```python
from build123d import *

# Parameters (mm, degrees)
EXTRUDE_1_DEPTH = 25


with BuildPart() as part:
    # 草图1 → 凸台-拉伸1 (new body)
    with BuildSketch(Plane(origin=(0, 0, 0), x_dir=(1, 0, 0), z_dir=(0, 1, 0))):
        Polygon((-115, 90), (-90, 115), (0, 115), (0, 0), (-115, 0), align=None)
    extrude(amount=EXTRUDE_1_DEPTH)


solid = part.part
```
Input: part model. Units: mm. Frame: model coordinates. Coordinates: 2 decimals unless noted, no trailing zeros. Loops run counter-clockwise (first coordinate to the right, second up) from the corner with the lowest first, then second, coordinate; pieces in that order, holes last. Notation, with made-up numbers: (27.5, -1) -> (55.5, -1) arc R23 ccw to (55.5, 14) -> close; hole circle Ø6 at (-2, 3.25). An arc over 180 degrees is marked (long way). Use a Markdown table: item, result.
1) Cut plane A-A (y = 9.5). Return the cut outline in (x, z), then the cut area to 3 significant figures.
Results found:
| item | result |
|---|---|
| outline | (-115, -90) -> (-90, -115) -> (0, -115) -> (0, 0) -> (-115, 0) -> close |
| area | 12,900 mm2 |
2) Material intervals for line 1 along X through (y, z) = (9, -97.5); line 2 along Z through (x, y) = (-107.5, 23.75); line 3 along X through (y, z) = (3, -95), sorted ascending. Write a range as from..to.
Results found:
| item | result |
|---|---|
| line 1 | x = -107.5..0 |
| line 2 | z = -97.5..0 |
| line 3 | x = -110..0 |
3) Contact query for a flat-ended pin moving along its axis: pin 1 (1 mm diameter, centred on x = -45.5, z = -96, fed in from -Y). Output: stop coordinate, or through.
Results found:
| item | result |
|---|---|
| pin 1 | stops at y = 0 |
4) Cut plane B-B (z = -98.5). Return the cut outline in (x, y), then the cut area to 3 significant figures.
Results found:
| item | result |
|---|---|
| outline | (-106.5, 0) -> (0, 0) -> (0, 25) -> (-106.5, 25) -> close |
| area | 2,660 mm2 |
